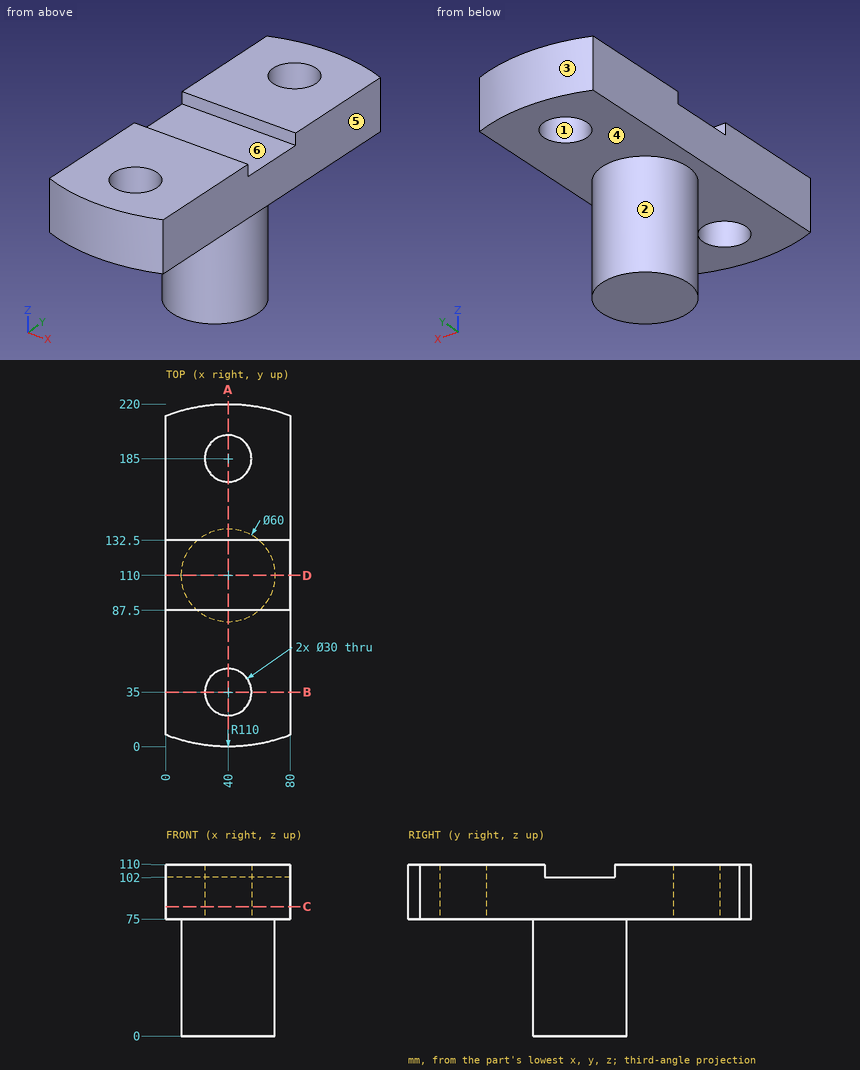
Geometry check sheet. Reference: drawing and pictorial views, mm from the part's lowest x, y, z. A direction names the side the tool comes from. Round coordinates to 2 decimals unless told otherwise and drop trailing zeros. Loops run counter-clockwise (first coordinate to the right, second up) from the corner with the lowest first, then second, coordinate; pieces in that order, holes last. Notation, with made-up numbers: (76, 71) -> (91, 71) arc R19 cw to (91, 81) -> close; hole circle Ø7 at (30, 44.5). An arc over 180 degrees is marked (long way). Answer as a JSON object with one key per item and string values. Group by question number.
Item 1: Cross-section at D-D, the plane y = 110. Record the cut outline in (x, z).
Item 2: Release check for a two-part mould opening along Y. For the marked faces 1, 2, 3 and 4 record: pulls with the +Y half, pulls with the -Y half, needs draft (parallel to the pull), parting line crosses it, or undercut.
Item 3: Cross-section at C-C, the plane z = 83. Record the cut outline in (x, y), plus the area to 3 significant figures.
Item 4: Depth check by flat-ended pin: pin 1 Ø2.5 at (x, z) = (58, 107.5) entering from -Y; pin 2 Ø2 at (x, y) = (70, 109) entering from +Z; pin 3 Ø8 at (x, z) = (18.5, 88) entering from -Y; pin 4 Ø24 at (x, y) = (40, 35) entering from +Z. Enter the tip coordinate at first touch or a pass-through.
Item 5: Thickness scan on line 1 along Y through (x, z) = (40, 90); line 2 along Y through (x, z) = (40, 102.5); line 3 along X through (y, z) = (35, 84). Record the ranges inside material, lowest first.
Item 6: Cross-section at A-A, the plane x = 40. Record the cut outline in (y, z), plus the area to 3 significant figures.
Item 7: Cross-section at B-B, the plane y = 35. Record the cut outline in (x, z).
Item 8: Set-up check for the marked faces 5 and 6: record each of +Z, -Z, +X, -X, +Y, -Y from which the full face is reachable in a straight line by a thin tool's end or side.
Determined:
{
 "1": {"outline": "(0, 75) -> (10, 75) -> (10, 0) -> (70, 0) -> (70, 75) -> (80, 75) -> (80, 102) -> (0, 102) -> close"},
 "2": {"face 1": "undercut", "face 2": "parting line crosses it", "face 3": "pulls with the +Y half", "face 4": "needs draft"},
 "3": {"outline": "(0, 7.53) arc R110 ccw to (80, 7.53) -> (80, 212.47) arc R110 ccw to (0, 212.47) -> close; hole circle Ø30 at (40, 35); hole circle Ø30 at (40, 185)", "area": "15,800 mm²"},
 "4": {"pin 1": "stops at y = 1.28", "pin 2": "stops at z = 102", "pin 3": "stops at y = 1.4", "pin 4": "passes through"},
 "5": {"line 1": "y = 0 to 20, 50 to 170, 200 to 220", "line 2": "y = 0 to 20, 50 to 87.5, 132.5 to 170, 200 to 220", "line 3": "x = 0 to 25, 55 to 80"},
 "6": {"outline": "(0, 75) -> (20, 75) -> (20, 110) -> (0, 110) -> close; (50, 75) -> (80, 75) -> (80, 0) -> (140, 0) -> (140, 75) -> (170, 75) -> (170, 110) -> (132.5, 110) -> (132.5, 102) -> (87.5, 102) -> (87.5, 110) -> (50, 110) -> close; (200, 75) -> (220, 75) -> (220, 110) -> (200, 110) -> close", "area": "9,740 mm²"},
 "7": {"outline": "(0, 75) -> (25, 75) -> (25, 110) -> (0, 110) -> close; (55, 75) -> (80, 75) -> (80, 110) -> (55, 110) -> close"},
 "8": {"face 5": "+Z, -Z, +X, +Y, -Y", "face 6": "+Z, +X, -X"}
}
